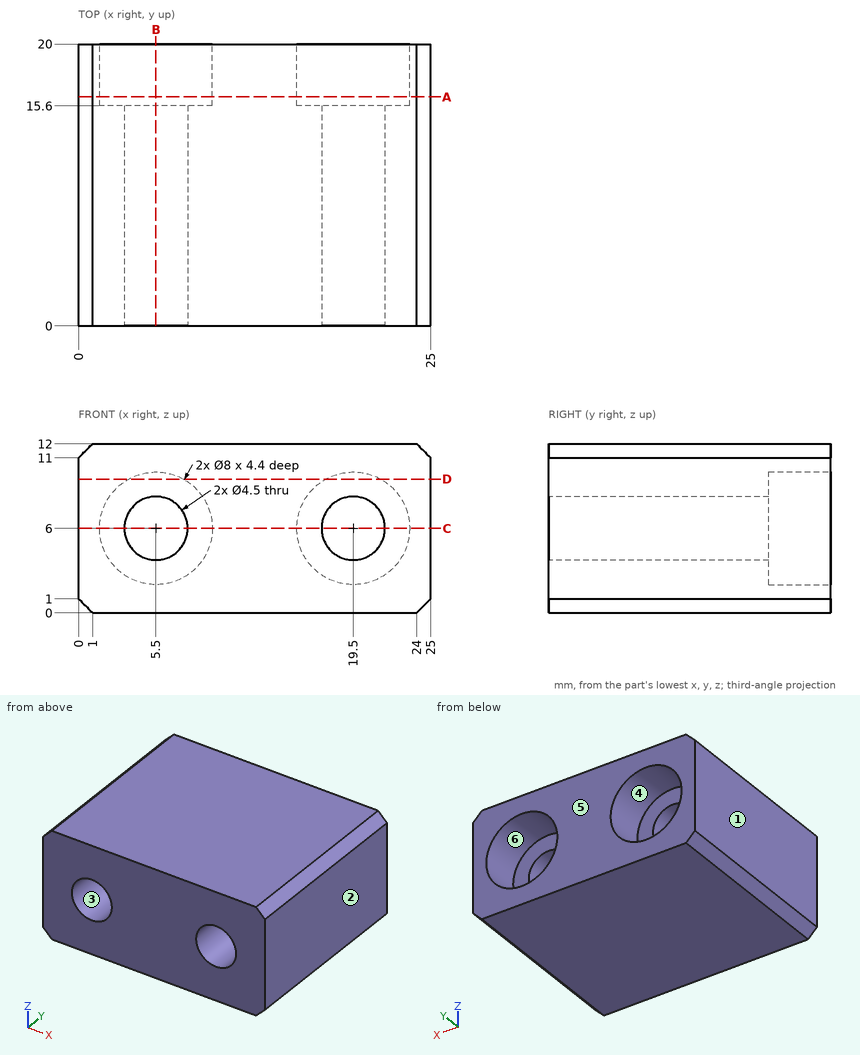
Drawing for the job (mm, zero at the part's lowest x, y, z). A direction names the side the tool comes from. Give positions to 0.01 mm unless a question says otherwise; leave off trailing zeros. Loops run counter-clockwise (first coordinate to the right, second up) from the corner with the lowest first, then second, coordinate; pieces in that order, holes last. Notation, with made-up numbers: M 87.5,83.25 L 96.5,83.25 A23 cw 96.5,100.25 Z; hole C 11.25,-0.5 d7. An arc over 180 degrees is marked long. Use one line per item in the form item = value.
Item 1: Slice it at B-B (x = 5.5). List the corners of the cut face in (y, z).
Determined:
outline = M 0,0 L 20,0 L 20,2 L 15.6,2 L 15.6,3.75 L 0,3.75 Z; M 0,8.25 L 15.6,8.25 L 15.6,10 L 20,10 L 20,12 L 0,12 Z
Item 2: Which spindle directions (+Z, -Z, +X, -X, +Y, -Y) get a long thin tool onto all of the face, cutting with end or side? Do the marked faces 5 and 6. Say none if no direction does.
Determined:
face_5 = +Z, -Z, +X, -X, +Y
face_6 = +Y
Item 3: Slice it at A-A (y = 16.25). List the corners of the cut face in (x, z).
Determined:
outline = M 0,1 L 1,0 L 24,0 L 25,1 L 25,11 L 24,12 L 1,12 L 0,11 Z; hole C 5.5,6 d8; hole C 19.5,6 d8
Item 4: Slice it at C-C (z = 6). List the corners of the cut face in (x, y), plus the area to 3 significant figures.
Determined:
outline = M 0,0 L 3.25,0 L 3.25,15.6 L 1.5,15.6 L 1.5,20 L 0,20 Z; M 7.75,0 L 17.25,0 L 17.25,15.6 L 15.5,15.6 L 15.5,20 L 9.5,20 L 9.5,15.6 L 7.75,15.6 Z; M 21.75,0 L 25,0 L 25,20 L 23.5,20 L 23.5,15.6 L 21.75,15.6 Z
area = 289 mm2
Item 5: Slice it at D-D (z = 9.5). List the corners of the cut face in (x, y), plus the area to 3 significant figures.
Determined:
outline = M 0,0 L 25,0 L 25,20 L 21.44,20 L 21.44,15.6 L 17.56,15.6 L 17.56,20 L 7.44,20 L 7.44,15.6 L 3.56,15.6 L 3.56,20 L 0,20 Z
area = 466 mm2
Item 6: Two-plate mould, pull along X, no slides. Class the marked faces 1, 2, 3 and 4: pulls with the +X half, pulls with the -X half, needs draft (parallel to the pull), parting line crosses it, or undercut.
Determined:
face_1 = pulls with the -X half
face_2 = pulls with the +X half
face_3 = undercut
face_4 = undercut
Item 7: Drill centre lines: probe 1 along Z at (x, y) = (5.5, 19.1); probe 2 along Z at (x, y) = (5.5, 13.5); probe 3 along X at (y, z) = (17, 3.5). Where is each one in solid material? Low to high. Write a range as from..to.
Determined:
probe_1 = 0..2, 10..12
probe_2 = 0..3.75, 8.25..12
probe_3 = 0..2.38, 8.62..16.38, 22.62..25
Item 8: Flat gauge pin, fed straight in: pin 1 (2.5 mm diameter, centred on x = 6, z = 5, fed in from +Y). Where does the tip first touch, or does it go through?
Determined:
pin_1 = 15.6
